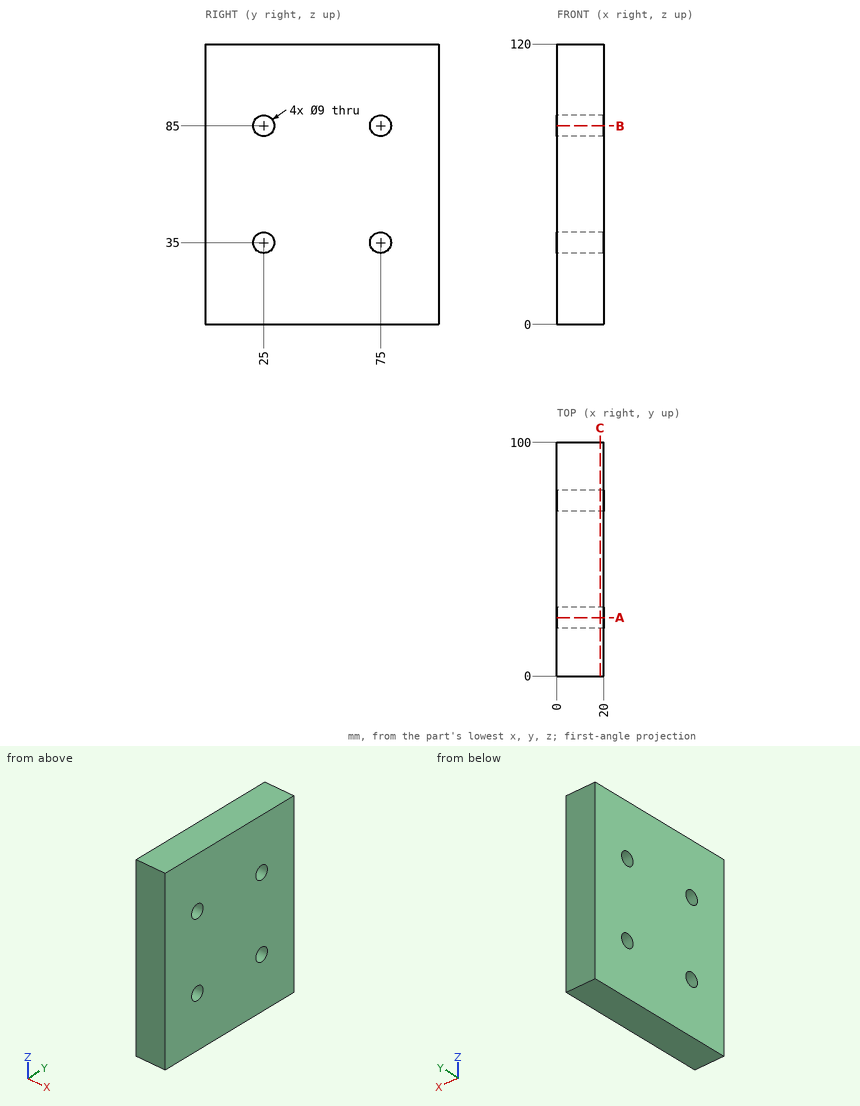
Answer from the drawing. Dimensions are ordinates in mm from the lowest x, y and z of the part. Coordinates: 2 decimals unless noted, no trailing zeros. Order: outer loops, then holes, each group sorted by start corner. A loop starts at its lowest first (then second) coordinate and runs counter-clockwise, first axis right, second up. Notation, with made-up numbers: (13.25, 48) - (38.25, 48) arc R18 ccw to (38.25, 65) - close; hole circle Ø6 at (22, 86). An arc over 180 degrees is marked (long way). Use one line per item in the form item = value.
(1) Section B-B, the plane z = 85 is taken. Give the vertices of the cut face in (x, y), then the cut area to 3 significant figures.
Computed values:
outline = (0, 0) - (20, 0) - (20, 20.5) - (0, 20.5) - close; (0, 29.5) - (20, 29.5) - (20, 70.5) - (0, 70.5) - close; (0, 79.5) - (20, 79.5) - (20, 100) - (0, 100) - close
area = 1,640 mm²
(2) Section C-C, the plane x = 18.5 is taken. Give the vertices of the cut face in (y, z), then the cut area to 3 significant figures.
Computed values:
outline = (0, 0) - (100, 0) - (100, 120) - (0, 120) - close; hole circle Ø9 at (25, 35); hole circle Ø9 at (25, 85); hole circle Ø9 at (75, 35); hole circle Ø9 at (75, 85)
area = 11,700 mm²
(3) Section A-A, the plane y = 25 is taken. Give the vertices of the cut face in (x, z), then the cut area to 3 significant figures.
Computed values:
outline = (0, 0) - (20, 0) - (20, 30.5) - (0, 30.5) - close; (0, 39.5) - (20, 39.5) - (20, 80.5) - (0, 80.5) - close; (0, 89.5) - (20, 89.5) - (20, 120) - (0, 120) - close
area = 2,040 mm²
(4) Given pin 1 Ø8 at (y, z) = (25, 85) entering from -X, flat-ended and moving along its own axis, determine where the tip first touches the part or whether it passes through.
Computed values:
pin_1 = through
(5) Straight lines are drawn through the part: L1, parallel to Y at x = 11.75, z = 85; L2, parallel to Y at x = 8.5, z = 87; L3, parallel to Z at x = 1.25, y = 77. For each, find the intervals that lie inside material, in ascending order.
Computed values:
L1 = 0 to 20.5, 29.5 to 70.5, 79.5 to 100
L2 = 0 to 20.97, 29.03 to 70.97, 79.03 to 100
L3 = 0 to 30.97, 39.03 to 80.97, 89.03 to 120
